CAD build for the part. Positions are in the model's coordinates, mm. Face numbers are marked on the shaded views. A direction names the side the tool comes from. Give positions to 0.01 mm unless a question says otherwise; leave off trailing zeros. Order: outer loops, then holes, each group sorted by start corner. A loop starts at its lowest first (then second) coordinate and runs counter-clockwise, first axis right, second up.
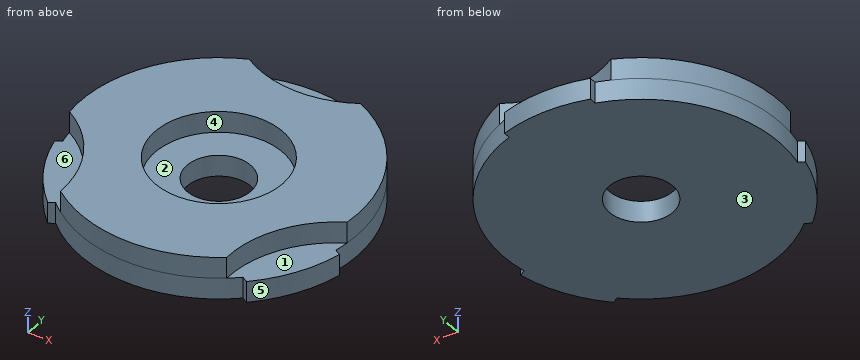
```python
from build123d import *

# Parameters (mm, degrees)
BASE_DISC_DEPTH       = 10
UPPER_SECTION_DEPTH   = 10
COUNTERBORE_SKETCH_R  = 30
COUNTERBORE_DEPTH     = 10
THROUGH_BORE_SKETCH_R = 15
THROUGH_BORE_DEPTH    = 10


with BuildPart() as part:
    # Base Disc Profile Sketch → Base Disc (new body)
    with BuildSketch(Plane.XY):
        with BuildLine():
            Line((20, 61.846584384), (20, 64.992307237))
            ThreePointArc((20, 64.992307237), (0, 68), (-20, 64.992307237))
            Line((-20, 64.992307237), (-20, 61.846584384))
            ThreePointArc((-20, 61.846584384), (-56.291651246, 32.5), (-63.560713214, -13.602784116))
            Line((-63.560713214, -13.602784116), (-66.284989118, -15.175645543))
            ThreePointArc((-66.284989118, -15.175645543), (-58.889727457, -34), (-46.284989118, -49.816661694))
            Line((-46.284989118, -49.816661694), (-43.560713214, -48.243800268))
            ThreePointArc((-43.560713214, -48.243800268), (0, -65), (43.560713214, -48.243800268))
            Line((43.560713214, -48.243800268), (46.284989118, -49.816661694))
            ThreePointArc((46.284989118, -49.816661694), (58.889727457, -34), (66.284989118, -15.175645543))
            Line((66.284989118, -15.175645543), (63.560713214, -13.602784116))
            ThreePointArc((63.560713214, -13.602784116), (56.291651246, 32.5), (20, 61.846584384))
        make_face()
    extrude(amount=BASE_DISC_DEPTH)

    # Upper Section Sketch → Upper Section (add)
    with BuildSketch(Plane.XY.offset(10)):
        with BuildLine():
            ThreePointArc((-25.892074701, 59.620470207), (-56.291651246, 32.5), (-64.578879135, -7.387040655))
            ThreePointArc((-64.578879135, -7.387040655), (-45.374794332, -26.197149722), (-38.686804434, -52.233429551))
            ThreePointArc((-38.686804434, -52.233429551), (0, -65), (38.686804434, -52.233429551))
            ThreePointArc((38.686804434, -52.233429551), (45.374794332, -26.197149722), (64.578879135, -7.387040655))
            ThreePointArc((64.578879135, -7.387040655), (56.291651246, 32.5), (25.892074701, 59.620470207))
            ThreePointArc((25.892074701, 59.620470207), (0, 52.394299444), (-25.892074701, 59.620470207))
        make_face()
    extrude(amount=UPPER_SECTION_DEPTH)

    # Counterbore Sketch → Counterbore (cut)
    with BuildSketch(Plane.XY.offset(20)):
        Circle(COUNTERBORE_SKETCH_R)
    extrude(amount=-COUNTERBORE_DEPTH, mode=Mode.SUBTRACT)

    # Through Bore Sketch → Through Bore (cut)
    with BuildSketch(Plane.XY.offset(10)):
        Circle(THROUGH_BORE_SKETCH_R)
    extrude(amount=-THROUGH_BORE_DEPTH, mode=Mode.SUBTRACT)


solid = part.part
```
Item 1: Slice it at C-C (x = 0). Give the cut face in (y, z), and give its area (3 significant figures).
Item 2: Slice it at D-D (z = 6.5). Give the cut face in (x, y).
Item 3: Slice it at B-B (y = 0). Give the cut face in (x, z), and give its area (3 significant figures).
Item 4: Wall check: L1, parallel to Y at x = 0, z = 3; L2, parallel to Y at x = 0, z = 18; L3, parallel to Z at x = -3.5, y = -22. Give the ranges that are in metal, low to high.
Item 5: Two-plate mould, pull along Y, no slides. Class the marked faces 4, 5 and 6: released by +Y, released by -Y, zero draft, split by the parting line, or undercut.
Item 6: Tool access for the marked faces 1, 2 and 3: list every direction of +Z, -Z, +X, -X, +Y, -Y with a clear straight run to the whole face (end or side of a thin tool).
Item 7: Slice it at A-A (z = 16). Give the cut face in (x, y).
Item 8: Drop flat-ended pins along their axis: pin 1 Ø2 at (x, z) = (-17.5, 2.5) entering from -Y; pin 2 Ø5 at (y, z) = (-29, 16.5) entering from +X; pin 3 Ø5 at (x, z) = (-12, 3.5) entering from -Y; pin 4 Ø18 at (x, y) = (0, 0) entering from +Z. Give the stop position or say it passes through.
A:
1. outline: (-65, 0) - (-15, 0) - (-15, 10) - (-30, 10) - (-30, 20) - (-65, 20) - close; (15, 0) - (68, 0) - (68, 10) - (52.39, 10) - (52.39, 20) - (30, 20) - (30, 10) - (15, 10) - close
1. area: 1,600 mm2
2. outline: (-66.28, -15.18) arc R68 ccw to (-46.28, -49.82) - (-43.56, -48.24) arc R65 ccw to (43.56, -48.24) - (46.28, -49.82) arc R68 ccw to (66.28, -15.18) - (63.56, -13.6) arc R65 ccw to (20, 61.85) - (20, 64.99) arc R68 ccw to (-20, 64.99) - (-20, 61.85) arc R65 ccw to (-63.56, -13.6) - close; hole circle Ø30 at (0, 0)
3. outline: (-65, 0) - (-15, 0) - (-15, 10) - (-30, 10) - (-30, 20) - (-65, 20) - close; (15, 0) - (65, 0) - (65, 20) - (30, 20) - (30, 10) - (15, 10) - close
3. area: 1,700 mm2
4. L1: y = -65 to -15, 15 to 68
4. L2: y = -65 to -30, 30 to 52.39
4. L3: z = 0 to 10
5. face 4: undercut
5. face 5: released by -Y
5. face 6: zero draft
6. face 1: +Z, +X, -Y
6. face 2: +Z
6. face 3: -Z, +X, -X, +Y, -Y
7. outline: (-64.58, -7.39) arc R50 cw to (-38.69, -52.23) arc R65 ccw to (38.69, -52.23) arc R50 cw to (64.58, -7.39) arc R65 ccw to (25.89, 59.62) arc R50 cw to (-25.89, 59.62) arc R65 ccw to start; hole circle Ø60 at (0, 0)
8. pin 1: stops at y = -62.87
8. pin 2: stops at x = 45.2
8. pin 3: stops at y = -64.3
8. pin 4: passes through
